Read the model definition and answer for the solid it produces. Units are mm, in the model's axes. A direction names the side the tool comes from. Coordinates: 2 decimals unless noted, no trailing zeros. Loops run counter-clockwise (first coordinate to the right, second up) from the corner with the lowest first, then second, coordinate; pieces in that order, holes last. Notation, with made-up numbers: (-4, 12.5) - (34, 12.5) arc R14 ccw to (34, 28.5) - close; hole circle Ø8 at (19, 5.5). An arc over 180 degrees is marked (long way). One line per item, written item: value. Start each with the question number.
from build123d import *

# Parameters (mm, degrees)
SKETCH1_R           = 2
BOSS_EXTRUDE1_DEPTH = 25
SKETCH2_W           = 15.41853157
SKETCH2_H           = 4
SKETCH2_W_2         = 11.817796653
CUT_EXTRUDE1_DEPTH  = 0.5
CHAMFER1_SIZE       = 0.5


with BuildPart() as part:
    # Sketch1 → Boss-Extrude1 (new, symmetric)
    with BuildSketch(Plane.XY):
        Circle(SKETCH1_R)
    extrude(amount=BOSS_EXTRUDE1_DEPTH, both=True)

    # Sketch2 → Cut-Extrude1 (cut)
    with BuildSketch(Plane(origin=(0, 2, 0), x_dir=(-1, 0, 0), z_dir=(0, 1, 0))):
        with Locations((0, 22)):
            Rectangle(SKETCH2_W, SKETCH2_H)
        with Locations((0.877102096, -22)):
            Rectangle(SKETCH2_W_2, SKETCH2_H)
    extrude(amount=-CUT_EXTRUDE1_DEPTH, mode=Mode.SUBTRACT)

    # Chamfer1
    chamfer1_edges = [part.edges().sort_by_distance(p)[0] for p in [
        (-2, 0, -25),
        (-2, 0, 25),
    ]]
    chamfer(chamfer1_edges, length=CHAMFER1_SIZE)


solid = part.part
1) Determine the mould class of faces 3 (the flat face through (0, 1.5, -22)), 4 (the flat face through (0, 0, 25)), 5 (the flat face through (0, 0, -25)) for opening direction Z: released by +Z, released by -Z, zero draft, split by the parting line, or undercut.
2) Straight lines are drawn through the part: L1, parallel to Z at x = -0.6, y = 1.8; L2, parallel to Y at x = -1.5, z = 1; L3, parallel to X at y = -0.2, z = -11. For each, find the intervals that lie inside material, in ascending order.
3) Flat-ended cylindrical pins translate along their axes: P1, Ø1.3, axis at x = 0, z = -22.5, coming from the +Y side; P2, Ø1.5, axis at x = 1.5, z = 13.5, coming from the -Y side; P3, Ø0.6, axis at x = -0.5, y = 2, coming from the +Z side; P4, Ø0.6, axis at x = -0.5, y = 1.5, coming from the -Z side. Find the tip coordinate at first contact, or state that the pin passes through.
4) Section B-B, the plane z = -6.5 is taken. Determine the outline of the cut face in (x, y), and give its area (3 significant figures).
5) Section C-C, the plane z = 21.5 is taken. Determine the outline of the cut face in (x, y), and give its area (3 significant figures).
6) For faces 1 (the cylindrical face through (0, -2, 0)), 2 (the flat face through (0, 1.5, 22)), determine the directions among +Z, -Z, +X, -X, +Y, -Y from which every point of the face is accessible in a straight line to the end or side of a thin tool.
7) Section A-A, the plane x = 0 is taken. Determine the outline of the cut face in (y, z), and give its area (4 significant figures).
Answer below:
1. face 3: undercut
1. face 4: released by +Z
1. face 5: released by -Z
2. L1: -24.6 to -24, -20 to 20, 24 to 24.6
2. L2: -1.32 to 1.32
2. L3: -1.99 to 1.99
3. P1: y = 1.5
3. P2: y = -1.85
3. P3: z = 24.74
3. P4: z = -25
4. outline: circle Ø4 at (0, 0)
4. area: 12.6 mm2
5. outline: (-1.32, 1.5) arc R2 ccw (long way) to (1.32, 1.5) - close
5. area: 11.7 mm2
6. face 1: +Z, -Z
6. face 2: +X, -X, +Y
7. outline: (-2, -24.5) - (-1.5, -25) - (1.5, -25) - (2, -24.5) - (2, -24) - (1.5, -24) - (1.5, -20) - (2, -20) - (2, 20) - (1.5, 20) - (1.5, 24) - (2, 24) - (2, 24.5) - (1.5, 25) - (-1.5, 25) - (-2, 24.5) - close
7. area: 195.5 mm2
